from build123d import *

# Parameters (mm, degrees)
SKETCH_1_W             = 8
SKETCH_1_H             = 120
HOLE_WIZARD_M6_1_D     = 5
HOLE_WIZARD_M6_1_DEPTH = 12
HOLE_WIZARD_M6_1_TIP   = 1.502151548
HOLE_WIZARD_M6_2_D     = 5
HOLE_WIZARD_M6_2_DEPTH = 12
HOLE_WIZARD_M6_2_TIP   = 1.502151548


with BuildPart() as part:
    # 草图1 → 旋转-薄壁1 (revolve)
    with BuildSketch(Plane.XY, mode=Mode.PRIVATE) as revolve_1_sk:
        with Locations((4, 0)):
            Rectangle(SKETCH_1_W, SKETCH_1_H)
    revolve(revolve_1_sk.sketch.rotate(Axis((0, 60, 0), (0, -1, 0)), 180), axis=Axis((0, 60, 0), (0, -1, 0)))

    # M6 螺纹孔的螺纹孔钻头1
    with Locations(Plane(origin=(0, 60, 0), x_dir=(1, 0, 0), z_dir=(0, 1, 0))):
        with Locations((0, 0)):
            Hole(HOLE_WIZARD_M6_1_D / 2, depth=HOLE_WIZARD_M6_1_DEPTH)
            with Locations((0, 0, -(HOLE_WIZARD_M6_1_DEPTH + HOLE_WIZARD_M6_1_TIP / 2))):  # 118° drill point
                Cone(0, HOLE_WIZARD_M6_1_D / 2, HOLE_WIZARD_M6_1_TIP, mode=Mode.SUBTRACT)

    # M6 螺纹孔的螺纹孔钻头2
    with Locations(Plane(origin=(0, -60, 0), x_dir=(-1, 0, 0), z_dir=(0, -1, 0))):
        with Locations((0, 0)):
            Hole(HOLE_WIZARD_M6_2_D / 2, depth=HOLE_WIZARD_M6_2_DEPTH)
            with Locations((0, 0, -(HOLE_WIZARD_M6_2_DEPTH + HOLE_WIZARD_M6_2_TIP / 2))):  # 118° drill point
                Cone(0, HOLE_WIZARD_M6_2_D / 2, HOLE_WIZARD_M6_2_TIP, mode=Mode.SUBTRACT)


solid = part.part
Source: CAD feature listing. Evaluate the final solid. Frame: model axes, mm. A direction names the side the tool comes from. Coordinates: 2 decimals unless noted, no trailing zeros. Order: outer loops, then holes, each group sorted by start corner. A loop starts at its lowest first (then second) coordinate and runs counter-clockwise, first axis right, second up. Notation, with made-up numbers: M 89.5,52 L 105.5,52 A34 ccw 105.5,91 Z; hole C 48.5,9 d2. An arc over 180 degrees is marked long. Write each question's results on one line, items separated by ' | '. Start each with the question number.
1. Material intervals for L1, parallel to Z at x = 0, y = 54.5; L2, parallel to Z at x = 1.5, y = -54.5; L3, parallel to Z at x = 0.25, y = -30, sorted ascending.
2. Section B-B, the plane z = -6. Return the cut outline in (x, y), then the cut area to 3 significant figures.
3. Draft query along X for faces 4 (the face through (2, -60, -2)), 5 (the face through (1.73, 0.84, 7.81)), 6 (the face through (0.094, -46.759, 0.424)). Return one class per face: +X half, -X half, draft (parallel to the pull), parting line (faces both ways), or undercut.
4. Pin query (flat end, axial travel): pin 1 (1.5 mm diameter, centred on x = -4.5, y = 32.5, fed in from +Z); pin 2 (4 mm diameter, centred on y = 40, z = -4.5, fed in from +X). Return the tip coordinate at first contact, or that it passes through.
5. Section A-A, the plane y = 9.5. Return the cut outline in (x, z), then the cut area to 3 significant figures.
6. Section C-C, the plane x = -4. Return the cut outline in (y, z).
7. Reachability of faces 1 (the face through (2, 60, -2)), 2 (the face through (-0.54, -53.92, 2.44)), 3 (the face through (0.54, 53.92, 2.44)) from +Z, -Z, +X, -X, +Y, -Y: full face, straight path, thin tool, end or side. Return the list, or none.
Solution:
1) L1: -8 to -2.5, 2.5 to 8 | L2: -7.86 to -2, 2 to 7.86 | L3: -8 to 8
2) outline: M -5.29,-60 L 5.29,-60 L 5.29,60 L -5.29,60 Z | area: 1,270 mm²
3) face 4: draft | face 5: parting line | face 6: undercut
4) pin 1: z = 7.07 | pin 2: x = 7.6
5) outline: C 0,0 d16 | area: 201 mm²
6) outline: M -60,-6.93 L 60,-6.93 L 60,6.93 L -60,6.93 Z
7) face 1: +Z, -Z, +X, -X, +Y | face 2: -Y | face 3: +Y
